from build123d import *

# Parameters (mm, degrees)
SKETCH1_R           = 6
BOSS_EXTRUDE1_DEPTH = 114.3
CHAMFER2_SIZE       = 0.9
BOSS_EXTRUDE2_DEPTH = 5


with BuildPart() as part:
    # Sketch1 → Boss-Extrude1 (new body)
    with BuildSketch(Plane.XY):
        Circle(SKETCH1_R)
    extrude(amount=BOSS_EXTRUDE1_DEPTH)

    # Chamfer2
    chamfer2_edges = [part.edges().sort_by_distance(p)[0] for p in [
        (-6, 0, 114.3),
    ]]
    chamfer(chamfer2_edges, length=CHAMFER2_SIZE)

    # Sketch2 → Boss-Extrude2 (add)
    with BuildSketch(Plane(origin=(0, 0, 0), x_dir=(-1, 0, 0), z_dir=(0, 0, -1))):
        with BuildLine():
            Line((11, 9.447221814), (11, -9.447221814))
            ThreePointArc((11, -9.447221814), (0, -14.5), (-11, -9.447221814))
            Line((-11, -9.447221814), (-11, 9.447221814))
            ThreePointArc((-11, 9.447221814), (0, 14.5), (11, 9.447221814))
        make_face()
    extrude(amount=BOSS_EXTRUDE2_DEPTH)


solid = part.part
Part model, mm, in its own coordinate system. A direction names the side the tool comes from. Give positions to 0.01 mm unless a question says otherwise; leave off trailing zeros. Loops run counter-clockwise (first coordinate to the right, second up) from the corner with the lowest first, then second, coordinate; pieces in that order, holes last.
(1) 3-axis set-ups, long thin cutter, end or side, ignore diameter. For faces 1 (the cylindrical face through (-6, 0, 56)), 2 (the flat face through (-11, 0, -2)): which of +Z, -Z, +X, -X, +Y, -Y reach the whole face in a straight line?
Return value:
face 1: +Z
face 2: +Z, -Z, -X, +Y, -Y
(2) Band-saw the part on A-A (x = 0). Write the cut outline in (y, z), and give its area (3 significant figures).
Return value:
outline: (-14.5, -5) - (14.5, -5) - (14.5, 0) - (6, 0) - (6, 113.4) - (5.1, 114.3) - (-5.1, 114.3) - (-6, 113.4) - (-6, 0) - (-14.5, 0) - close
area: 1,520 mm2
(3) Band-saw the part on C-C (z = 105). Write the cut outline in (x, y).
Return value:
outline: circle Ø12 at (0, 0)
(4) Drill centre lines: line 1 along Z through (x, y) = (5, -11.5); line 2 along Y through (x, z) = (0, 31); line 3 along X through (y, z) = (5.5, 103.5). Where is each one in solid material? Low to high.
Return value:
line 1: z = -5 to 0
line 2: y = -6 to 6
line 3: x = -2.4 to 2.4
(5) Band-saw the part on B-B (y = 0). Write the cut outline in (x, z), and give its area (3 significant figures).
Return value:
outline: (-11, -5) - (11, -5) - (11, 0) - (6, 0) - (6, 113.4) - (5.1, 114.3) - (-5.1, 114.3) - (-6, 113.4) - (-6, 0) - (-11, 0) - close
area: 1,480 mm2
(6) Band-saw the part on D-D (y = -7). Write the cut outline in (x, z).
Return value:
outline: (-11, -5) - (11, -5) - (11, 0) - (-11, 0) - close
(7) Pin check, flat tips, straight feed: pin 1 (4 mm diameter, centred on x = -3, z = 88.5, fed in from +Y); pin 2 (3 mm diameter, centred on y = 1.5, z = 18.5, fed in from -X); pin 3 (2 mm diameter, centred on x = -4.5, y = -8.5, fed in from +Z); pin 4 (12 mm diameter, centred on x = -0.5, y = 7, fed in from +Z). Stop position of each tip, or through.
Return value:
pin 1: stops at y = 5.92
pin 2: stops at x = -6
pin 3: stops at z = 0
pin 4: stops at z = 114.3
